Model file for the job. Use its own axes, mm. A direction names the side the tool comes from. Coordinates: 2 decimals unless noted, no trailing zeros. Write each loop counter-clockwise with the first axis right and the second up, starting at its lowest first coordinate (ties: lowest second). Pieces come first, ordered by that corner, then holes. Notation, with made-up numbers: M 63.25,47.25 L 82.25,47.25 A28 ccw 82.25,83.25 Z; hole C 80,-36 d5. An arc over 180 degrees is marked long. One line per question, with ' | ' between items. Start each with the question number.
(1) Two-plate mould, pull along X, no slides. Class faces 1 (the face through (-39, 20, 0)), 2 (the face through (14.564, 3.944, 14.807)), 3 (the face through (-1, 31, -9.5)): +X half, -X half, draft (parallel to the pull), parting line (faces both ways), or undercut.
(2) Tool access for faces 4 (the face through (-3.14, 45.65, -39.46)), 5 (the face through (31.334, 33.124, -35.234)), 6 (the face through (-32, 15, 0)): list every direction of +Z, -Z, +X, -X, +Y, -Y with a clear straight run to the whole face (end or side of a thin tool).
(3) Cut at A-A (x = -8.5). Write the cut outline in (y, z), plus the area to 3 significant figures.
(4) Cut at C-C (y = 15.5). Write the cut outline in (x, z), plus the area to 3 significant figures.
(5) Cut at D-D (z = -15). Write the cut outline in (x, y), plus the area to 3 significant figures.
(6) Flat gauge pins, fed straight in: pin 1 Ø7.5 at (x, y) = (-4.5, 52.5) entering from +Z; pin 2 Ø16 at (x, z) = (-19, 12.5) entering from +Y; pin 3 Ø5 at (x, z) = (-28, -32) entering from -Y; pin 4 Ø6 at (x, z) = (19, 12.5) entering from -Y. Where does each tip first touch, or does it go through?
(7) Cut at B-B (z = 12.5). Write the cut outline in (x, y), plus the area to 3 significant figures.
(8) Wall check: probe 1 along X at (y, z) = (3, 12); probe 2 along Z at (x, y) = (-25.5, 8.5); probe 3 along Z at (x, y) = (7.5, 5.5). Give the ranges that are in metal, low to high.
from build123d import *

# Parameters (mm, degrees)
BASE_PLATE_SKETCH_W                  = 78
BASE_PLATE_SKETCH_H                  = 41
BASE_PLATE_SKETCH_R                  = 5
BASE_PLATE_WITH_MOUNTING_HOLES_DEPTH = 8
UPRIGHT_WALL_SKETCH_W                = 7
UPRIGHT_WALL_SKETCH_H                = 41
UPRIGHT_WALL_DEPTH                   = 38
BACK_PLATE_SKETCH_W                  = 78
BACK_PLATE_SKETCH_H                  = 7
BACK_PLATE_DEPTH                     = 82
WALL_TRIM_CUT_DEPTH                  = 58
ANGLED_TRIM_CUT_25DEG_DEPTH          = 58
INCLINED_FLANGE_DEPTH                = 38
FLANGE_PROFILE_CUT_SKETCH_W          = 9.958327832
FLANGE_PROFILE_CUT_SKETCH_H          = 38
FLANGE_PROFILE_CUT_SKETCH_W_2        = 7
FLANGE_PROFILE_CUT_DEPTH             = 38
KEYHOLE_SLOT_DIA18_X_W8_REACH        = 92.402


with BuildPart() as part:
    # Base Plate Sketch → Base Plate with Mounting Holes (new body)
    with BuildSketch(Plane(origin=(0, 0, 0), x_dir=(1, 0, 0), z_dir=(0, 1, 0))):
        with Locations((0, -4)):
            Rectangle(BASE_PLATE_SKETCH_W, BASE_PLATE_SKETCH_H)
        with Locations(Location((-19, -12.5, 0), (0, 0, 270))):
            Circle(BASE_PLATE_SKETCH_R, mode=Mode.SUBTRACT)
        with Locations(Location((19, -12.5, 0), (0, 0, 270))):
            Circle(BASE_PLATE_SKETCH_R, mode=Mode.SUBTRACT)
    extrude(amount=BASE_PLATE_WITH_MOUNTING_HOLES_DEPTH)

    # Upright Wall Sketch → Upright Wall (add)
    with BuildSketch(Plane(origin=(0, 8, 0), x_dir=(1, 0, 0), z_dir=(0, 1, 0))):
        with Locations((-35.5, -4)):
            Rectangle(UPRIGHT_WALL_SKETCH_W, UPRIGHT_WALL_SKETCH_H)
    extrude(amount=UPRIGHT_WALL_DEPTH)

    # Back Plate Sketch → Back Plate (add)
    with BuildSketch(Plane(origin=(0, 8, 0), x_dir=(1, 0, 0), z_dir=(0, 1, 0))):
        with Locations((0, 13)):
            Rectangle(BACK_PLATE_SKETCH_W, BACK_PLATE_SKETCH_H)
    extrude(amount=BACK_PLATE_DEPTH)

    # Wall Trim Sketch → Wall Trim Cut (cut)
    with BuildSketch(Plane(origin=(-32, 0, 0), x_dir=(0, 0, -1), z_dir=(1, 0, 0))):
        Polygon((9.5, 33), (-24.5, 8), (-24.5, 46), (9.5, 46), align=None)
    extrude(amount=-WALL_TRIM_CUT_DEPTH, mode=Mode.SUBTRACT)

    # Angled Trim Sketch 25deg → Angled Trim Cut 25deg (cut)
    with BuildSketch(Plane.XY.offset(-9.5)):
        Polygon((-39, 69.371997336), (39, 33), (39, 90), (-39, 90), align=None)
    extrude(amount=-ANGLED_TRIM_CUT_25DEG_DEPTH, mode=Mode.SUBTRACT)

    # Inclined Flange Sketch → Inclined Flange (add)
    with BuildSketch(Plane(origin=(0, 0, -16.5), x_dir=(-1, 0, 0), z_dir=(0, 0, -1))):
        Polygon((-39, 33), (39, 69.371997336), (39, 62.371997336), (-39, 26), align=None)
    extrude(amount=INCLINED_FLANGE_DEPTH)

    # Flange Profile Cut Sketch → Flange Profile Cut (cut)
    with BuildSketch(Plane(origin=(19.605374923, 42.043862201, 0), x_dir=(0.9063077870366495, -0.42261826174070033, 0), z_dir=(0.42261826174070033, 0.9063077870366495, 0))):
        with Locations((19.378764973, 35.5)):
            Rectangle(FLANGE_PROFILE_CUT_SKETCH_W, FLANGE_PROFILE_CUT_SKETCH_H)
        with Locations((-61.163876622, 35.5)):
            Rectangle(FLANGE_PROFILE_CUT_SKETCH_W_2, FLANGE_PROFILE_CUT_SKETCH_H)
    extrude(amount=-FLANGE_PROFILE_CUT_DEPTH, mode=Mode.SUBTRACT)

    # Keyhole Slot Sketch → Keyhole Slot Dia18 x W8 (cut, up to next)
    with BuildSketch(Plane(origin=(19.605374923, 42.043862201, 0), x_dir=(0.9063077870366495, -0.42261826174070033, 0), z_dir=(0.42261826174070033, 0.9063077870366495, 0)), mode=Mode.PRIVATE) as keyhole_slot_dia18_x_w8_sk1:
        with BuildLine():
            Line((-35.600398943, 38.5), (-13.662656691, 38.5))
            ThreePointArc((-13.662656691, 38.5), (3.399601057, 34.5), (-13.662656691, 30.5))
            Line((-13.662656691, 30.5), (-35.600398943, 30.5))
            ThreePointArc((-35.600398943, 30.5), (-39.600398943, 34.5), (-35.600398943, 38.5))
        make_face()
    keyhole_slot_dia18_x_w8_tool1 = extrude(keyhole_slot_dia18_x_w8_sk1.sketch, amount=-KEYHOLE_SLOT_DIA18_X_W8_REACH, mode=Mode.PRIVATE) & part.part
    add(keyhole_slot_dia18_x_w8_tool1.solids().sort_by_distance((6.285215, 48.255155, -34.5))[0], mode=Mode.SUBTRACT)


solid = part.part
Filled in:
1) face 1: -X half | face 2: undercut | face 3: draft
2) face 4: -Z, -X, -Y | face 5: -Z, +X, -Y | face 6: +Z, +X, +Y
3) outline: M 0,-16.5 L 48.15,-16.5 L 48.15,-30.5 L 55.15,-30.5 L 55.15,-9.5 L 8,-9.5 L 8,24.5 L 0,24.5 Z; M 48.15,-54.5 L 55.15,-54.5 L 55.15,-38.5 L 48.15,-38.5 Z | area: 868 mm²
4) outline: M -39,-16.5 L 39,-16.5 L 39,-9.5 L -32,-9.5 L -32,14.3 L -39,14.3 Z | area: 713 mm²
5) outline: M -39,0 L 39,0 L 39,33 L -39,69.37 Z | area: 3,990 mm²
6) pin 1: z = -9.5 | pin 2: y = 8 | pin 3: y = 56.08 | pin 4: through
7) outline: M -39,0 L -24,0 L -24,8 L -32,8 L -32,16.82 L -39,16.82 Z; M -14,0 L 14,0 L 14,8 L -14,8 Z; M 24,0 L 39,0 L 39,8 L 24,8 Z | area: 526 mm²
8) probe 1: -39 to -23.97, -14.03 to 14.03, 23.97 to 39 | probe 2: -16.5 to -9.5 | probe 3: -16.5 to 24.5
